```python
from build123d import *

# Parameters (mm, degrees)
LINK_PROFILE_SKETCH_R = 5
LINK_PLATE_5MM_DEPTH  = 5


with BuildPart() as part:
    # Link Profile Sketch → Link Plate 5mm (new body)
    with BuildSketch(Plane(origin=(0, 0, 0), x_dir=(1, 0, 0), z_dir=(0, 1, 0))):
        with BuildLine():
            Line((-50, 10), (50, 10))
            ThreePointArc((50, 10), (60, 0), (50, -10))
            Line((50, -10), (-50, -10))
            ThreePointArc((-50, -10), (-60, 0), (-50, 10))
        make_face()
        with Locations(Location((-50, 0, 0), (0, 0, 270))):
            Circle(LINK_PROFILE_SKETCH_R, mode=Mode.SUBTRACT)
        with Locations(Location((50, 0, 0), (0, 0, 270))):
            Circle(LINK_PROFILE_SKETCH_R, mode=Mode.SUBTRACT)
        with BuildLine():
            Line((-35, 5), (35, 5))
            ThreePointArc((35, 5), (40, 0), (35, -5))
            Line((35, -5), (-35, -5))
            ThreePointArc((-35, -5), (-40, 0), (-35, 5))
        make_face(mode=Mode.SUBTRACT)
    extrude(amount=LINK_PLATE_5MM_DEPTH)


solid = part.part
```
Here's how the part is built. I have some questions about the finished solid (model axes, mm). A direction names the side the tool comes from. Round coordinates to 2 decimals unless told otherwise and drop trailing zeros. Order: outer loops, then holes, each group sorted by start corner. A loop starts at its lowest first (then second) coordinate and runs counter-clockwise, first axis right, second up. Notation, with made-up numbers: (-25.5, 37.5) -> (-10.5, 37.5) arc R14 cw to (-10.5, 49.5) -> close; hole circle Ø4 at (3, 56). An arc over 180 degrees is marked (long way). Use a Markdown table: item, result. Add a question column.
(1) For faces 1 (the face through (60, 2, 0)), 2 (the face through (0, 2, -5)), which set-ups out of +Z, -Z, +X, -X, +Y, -Y let a thin tool reach every point of the face, with its end or its side?
(2) Suppose I cut it at C-C, the plane x = -36. Please give me the cut outline in (y, z), and give its area (3 significant figures).
(3) Suppose I cut it at D-D, the plane z = 8. Please give me the cut outline in (x, y).
(4) If we mould it in two halves opening along Z, with no side actions, what happens to faces 3 (the face through (40, 2, 0)), 4 (the face through (1, 0, -7)), 5 (the face through (-60, 2, 0)), 6 (the face through (-1, 2, -10))? For each: released by +Z, released by -Z, zero draft, split by the parting line, or undercut.
(5) For pin 1 Ø5 at (x, z) = (35, -0.5) entering from -Y; pin 2 Ø2 at (y, z) = (2.5, 5) entering from +X, each with a flat end and sliding along its axis, tell me the tip position at first contact or that it passes through.
(6) Suppose I cut it at A-A, the plane z = 0. Please give me the cut outline in (x, y).
(7) Suppose I cut it at B-B, the plane y = 2.5. Please give me the cut outline in (x, z).
(8) I need wall thicknesses on line 1 along X through (y, z) = (1.5, 0); line 2 along Z through (x, y) = (-5, 3.9); line 3 along X through (y, z) = (1.35, 4). Which ranges of each line are inside material? Lowest first, please.
Verdict:
| question | item | result |
|---|---|---|
| 1 | face 1 | +X, +Y, -Y |
| 1 | face 2 | +Y, -Y |
| 2 | outline | (0, -10) -> (5, -10) -> (5, -4.9) -> (0, -4.9) -> close; (0, 4.9) -> (5, 4.9) -> (5, 10) -> (0, 10) -> close |
| 2 | area | 51.0 mm2 |
| 3 | outline | (-56, 0) -> (56, 0) -> (56, 5) -> (-56, 5) -> close |
| 4 | face 3 | undercut |
| 4 | face 4 | zero draft |
| 4 | face 5 | split by the parting line |
| 4 | face 6 | released by -Z |
| 5 | pin 1 | through |
| 5 | pin 2 | x = 59.17 |
| 6 | outline | (-60, 0) -> (-55, 0) -> (-55, 5) -> (-60, 5) -> close; (-45, 0) -> (-40, 0) -> (-40, 5) -> (-45, 5) -> close; (40, 0) -> (45, 0) -> (45, 5) -> (40, 5) -> close; (55, 0) -> (60, 0) -> (60, 5) -> (55, 5) -> close |
| 7 | outline | (-50, -10) -> (50, -10) arc R10 ccw to (50, 10) -> (-50, 10) arc R10 ccw to start; hole circle Ø10 at (-50, 0); hole (-35, -5) -> (35, -5) arc R5 ccw to (35, 5) -> (-35, 5) arc R5 ccw to start; hole circle Ø10 at (50, 0) |
| 8 | line 1 | -60 to -55, -45 to -40, 40 to 45, 55 to 60 |
| 8 | line 2 | -10 to -5, 5 to 10 |
| 8 | line 3 | -59.17 to -53, -47 to -38, 38 to 47, 53 to 59.17 |
